from build123d import *

# Parameters (mm, degrees)
EXTRUDE_1_DEPTH = 85
SKETCH_4_W      = 14
SKETCH_4_H      = 35
EXTRUDE_2_DEPTH = 45


with BuildPart() as part:
    # 草图1 → 凸台-拉伸1 (new, symmetric)
    with BuildSketch(Plane.XY):
        Polygon((0, 0), (0, 172), (14, 172), (14, 147), (12.5, 147), (12.5, 0), align=None)
    extrude(amount=EXTRUDE_1_DEPTH, both=True)

    # 草图4 → 凸台-拉伸2 (add)
    with BuildSketch(Plane(origin=(0, 0, -85), x_dir=(-1, 0, 0), z_dir=(0, 0, -1))):
        with Locations((-7, 126)):
            Rectangle(SKETCH_4_W, SKETCH_4_H)
    extrude(amount=EXTRUDE_2_DEPTH)


solid = part.part
Geometry check sheet. Reference: the model listing, model coordinates, mm. A direction names the side the tool comes from. Give positions to 0.01 mm unless a question says otherwise; leave off trailing zeros. Order: outer loops, then holes, each group sorted by start corner. A loop starts at its lowest first (then second) coordinate and runs counter-clockwise, first axis right, second up.
1) Cross-section at D-D (y = 27). Record the boundary of the cut face in (x, z).
Results are:
outline: (0, -85) - (12.5, -85) - (12.5, 85) - (0, 85) - close
2) Material ranges on probe 1 along Z at (x, y) = (7.5, 73); probe 2 along X at (y, z) = (27, 63.5); probe 3 along Y at (x, z) = (4.25, -108), recorded low to high.
Results are:
probe 1: z = -85 to 85
probe 2: x = 0 to 12.5
probe 3: y = 108.5 to 143.5
3) Tool access check on faces 1 (the flat face through (7, 158, -85)), 2 (the flat face through (7, 108.5, -107)), 3 (the flat face through (12.5, 75, 1)), 4 (the flat face through (7, 87, 85)), 5 (the flat face through (6, 0, 1)). Record the directions out of +Z, -Z, +X, -X, +Y, -Y that give a thin tool (end or side, any length) a straight path to the whole face; none if there is none.
Results are:
face 1: -Z, +X, -X, +Y
face 2: -Z, +X, -X, -Y
face 3: +Z, +X, -Y
face 4: +Z, +X, -X, +Y, -Y
face 5: +Z, -Z, +X, -X, -Y
4) Cross-section at A-A (x = 3.25). Record the boundary of the cut face in (y, z), then the cut area to 3 significant figures.
Results are:
outline: (0, -85) - (108.5, -85) - (108.5, -130) - (143.5, -130) - (143.5, -85) - (172, -85) - (172, 85) - (0, 85) - close
area: 30,800 mm2
5) Cross-section at C-C (y = 135). Record the boundary of the cut face in (x, z).
Results are:
outline: (0, -130) - (14, -130) - (14, -85) - (12.5, -85) - (12.5, 85) - (0, 85) - close
6) Gauge pin test, flat ends, axial feed: pin 1 (2 mm diameter, centred on x = 7, z = -100.5, fed in from +Y); pin 2 (1.6 mm diameter, centred on x = 13.5, y = 134, fed in from +Z); pin 3 (6 mm diameter, centred on x = 6.5, y = 59.5, fed in from -Z). Record the tip position at first contact, or that the pin passes through.
Results are:
pin 1: stops at y = 143.5
pin 2: stops at z = -85
pin 3: stops at z = -85
7) Cross-section at B-B (z = -13). Record the boundary of the cut face in (x, y), then the cut area to 3 significant figures.
Results are:
outline: (0, 0) - (12.5, 0) - (12.5, 147) - (14, 147) - (14, 172) - (0, 172) - close
area: 2,190 mm2
